Input: dimensioned drawing with shaded views. Units: mm. Origin: part minimum x, y, z. A direction names the side the tool comes from. Coordinates: 2 decimals unless noted, no trailing zeros. Write each loop counter-clockwise with the first axis right and the second up, starting at its lowest first coordinate (ties: lowest second). Pieces come first, ordered by that corner, then holes. Notation, with made-up numbers: M 70,27.5 L 97,27.5 A9 cw 97,44.5 Z; hole C 16.25,-14.5 d7. An arc over 180 degrees is marked long. Use one line per item in the form item = value.
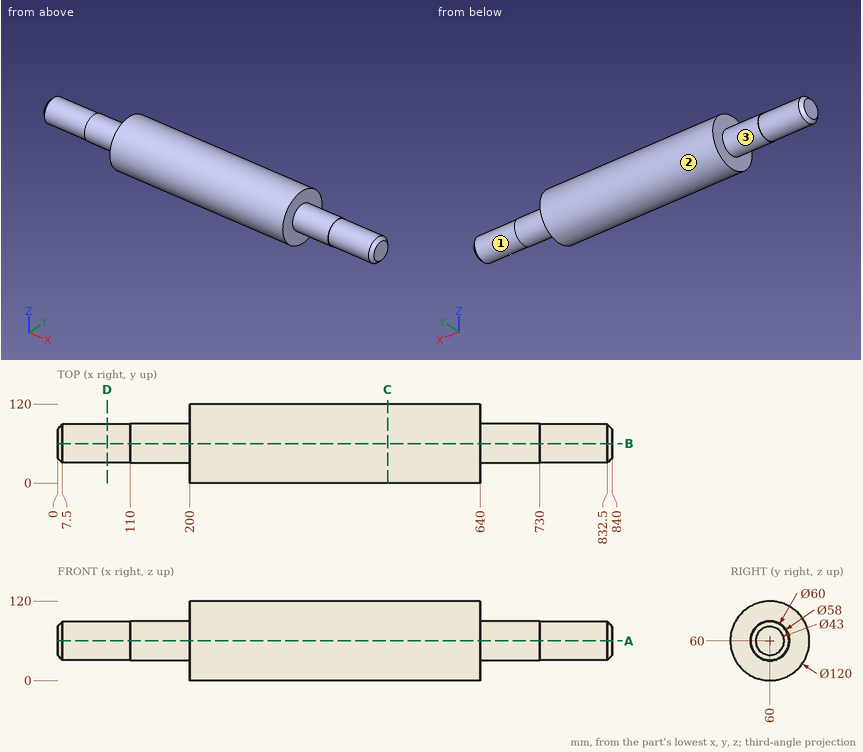
(1) Section query A-A on z = 60. Return the cut outline in (x, y).
Computed:
outline = M 0,38.5 L 7.5,31 L 110,31 L 110,30 L 200,30 L 200,0 L 640,0 L 640,30 L 730,30 L 730,31 L 832.5,31 L 840,38.5 L 840,81.5 L 832.5,89 L 730,89 L 730,90 L 640,90 L 640,120 L 200,120 L 200,90 L 110,90 L 110,89 L 7.5,89 L 0,81.5 Z
(2) First-contact query: pin 1 Ø2 at (y, z) = (24.5, 69) entering from -X; pin 2 Ø12 at (x, z) = (472.5, 93.5) entering from -Y; pin 3 Ø10 at (x, y) = (567.5, 89.5) entering from -Z. Flat tips, straight axial feed; report the tip coordinate or a pass-through.
Computed:
pin_1 = 200
pin_2 = 6.67
pin_3 = 5.23
(3) Section query D-D on x = 75. Return the cut outline in (y, z).
Computed:
outline = C 60,60 d58
(4) Section query C-C on x = 500. Return the cut outline in (y, z).
Computed:
outline = C 60,60 d120
(5) Line query: probe 1 along Z at (x, y) = (654, 59); probe 2 along X at (y, z) = (52.5, 90); probe 3 along Z at (x, y) = (438.5, 61.5). Output: solid intervals per line, ascending.
Computed:
probe_1 = 30.02 to 89.98
probe_2 = 200 to 640
probe_3 = 0.02 to 119.98
(6) Set-up query: the marked faces 1, 2 and 3. Return all of +Z, -Z, +X, -X, +Y, -Y with unobstructed straight access to the full face (end or side cutting, diameter ignored); none if empty.
Computed:
face_1 = +X
face_2 = +X, -X
face_3 = -X
